Geometry check sheet. Reference: drawing and pictorial views, mm from the part's lowest x, y, z. A direction names the side the tool comes from. Give positions to 0.01 mm unless a question says otherwise; leave off trailing zeros. Order: outer loops, then holes, each group sorted by start corner. A loop starts at its lowest first (then second) coordinate and runs counter-clockwise, first axis right, second up. Notation, with made-up numbers: M 0.5,88 L 50.5,88 A28 cw 50.5,111 Z; hole C -6.75,76 d6. An arc over 180 degrees is marked long. Answer as CSV lines item,"result". Start each with the question number.
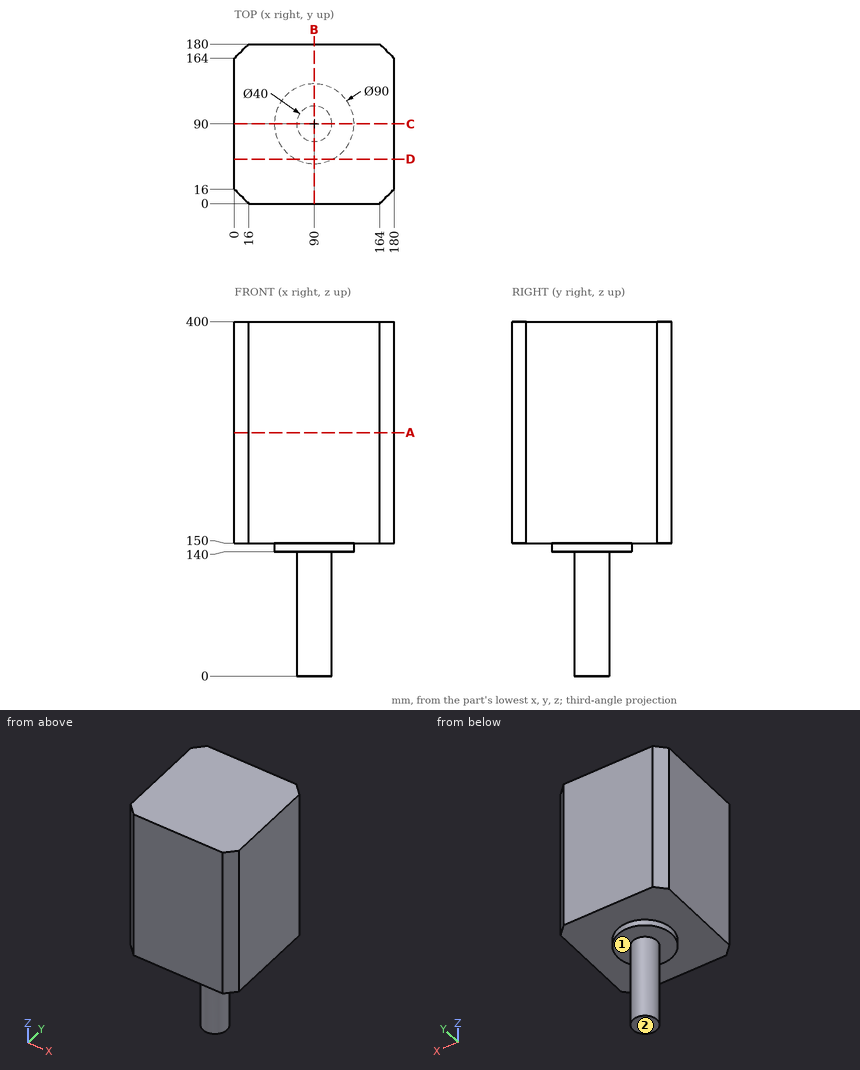
Item 1: Scan lines: line 1 along Z through (x, y) = (123, 38); line 2 along Z through (x, y) = (83.5, 46.5); line 3 along X through (y, z) = (80, 20.5). Record each from-to range of solid material in increasing order.
Item 2: Section check A-A on z = 274.5. Record the boundary of the cut face in (x, y), then the cut area to 3 significant figures.
Item 3: Section check B-B on x = 90. Record the boundary of the cut face in (y, z), then the cut area to 3 significant figures.
Item 4: Depth check by flat-ended pin: pin 1 Ø5 at (y, z) = (103, 132) entering from -X; pin 2 Ø5 at (x, y) = (124.5, 117.5) entering from -Z; pin 3 Ø10 at (x, z) = (66.5, 75.5) entering from -Y. Enter the tip coordinate at first touch or a pass-through.
Item 5: Section check D-D on y = 50. Record the boundary of the cut face in (x, z).
Item 6: Access from +Z, -Z, +X, -X, +Y, -Y to the whole of each face (thin tool, end or side, straight path). Record for the marked faces 1 and 2.
Numbers:
1,line 1,"150 to 400"
1,line 2,"140 to 400"
1,line 3,"72.68 to 107.32"
2,outline,"M 0,16 L 16,0 L 164,0 L 180,16 L 180,164 L 164,180 L 16,180 L 0,164 Z"
2,area,"31,900 mm2"
3,outline,"M 0,150 L 45,150 L 45,140 L 70,140 L 70,0 L 110,0 L 110,140 L 135,140 L 135,150 L 180,150 L 180,400 L 0,400 Z"
3,area,"51,500 mm2"
4,pin 1,"x = 72.98"
4,pin 2,"z = 140"
4,pin 3,"y = 82.4"
5,outline,"M 0,150 L 69.38,150 L 69.38,140 L 110.62,140 L 110.62,150 L 180,150 L 180,400 L 0,400 Z"
6,face 1,"-Z"
6,face 2,"-Z, +X, -X, +Y, -Y"
